```python
from build123d import *

# Parameters (mm, degrees)
SKETCH_1_R      = 4
EXTRUDE_1_DEPTH = 140
EXTRUDE_START   = -20
SKETCH_2_R      = 7.5
EXTRUDE_2_DEPTH = 5
EXTRUDE_START_2 = -15
SKETCH_3_R      = 7.5
EXTRUDE_3_DEPTH = 5


with BuildPart() as part:
    # 草图1 → 凸台-拉伸1 (new, symmetric)
    with BuildSketch(Plane.XY):
        Circle(SKETCH_1_R)
    extrude(amount=EXTRUDE_1_DEPTH, both=True)

    # 草图2 → 凸台-拉伸2 (add)
    with BuildSketch(Plane.XY.offset(140).offset(EXTRUDE_START)):
        Circle(SKETCH_2_R)
    extrude(amount=-EXTRUDE_2_DEPTH)

    # 草图3 → 凸台-拉伸3 (add)
    with BuildSketch(Plane(origin=(0, 0, -140), x_dir=(-1, 0, 0), z_dir=(0, 0, -1)).offset(EXTRUDE_START_2)):
        with Locations(Location((0, 0, 0), (0, 0, 180))):
            Circle(SKETCH_3_R)
    extrude(amount=EXTRUDE_3_DEPTH)


solid = part.part
```
Geometry: final body of the model. Coordinates: model frame, mm. A direction names the side the tool comes from. Coordinates: 2 decimals unless noted, no trailing zeros. Order: outer loops, then holes, each group sorted by start corner. A loop starts at its lowest first (then second) coordinate and runs counter-clockwise, first axis right, second up. Notation, with made-up numbers: M -14,39 L 22,39 A22 ccw 22,68 Z; hole C 44,65 d6. An arc over 180 degrees is marked long. Answer in a Markdown table with one row per item. Add a question column.
Q1. Mould query, pull axis Z, two halves, no side actions, for faces 5 (the flat face through (3, 3, -130)), 6 (the cylindrical face through (4.032, -6.324, -127.465)), 7 (the flat face through (3, -3, 115)). Classes: released by +Z, released by -Z, zero draft, split by the parting line, or undercut.
Q2. Reachability of faces 1 (the cylindrical face through (-0.867, -3.905, 130.14)), 2 (the cylindrical face through (-0.867, -3.905, -134.93)), 3 (the cylindrical face through (-0.867, -3.905, -3.32)), 4 (the flat face through (0, 0, 140)) from +Z, -Z, +X, -X, +Y, -Y: full face, straight path, thin tool, end or side. Return the list, or none.
Q3. Section query A-A on x = 0. Return the cut outline in (y, z), and give its area (3 significant figures).
Q4. Line query: L1, parallel to Z at x = 5.25, y = 0; L2, parallel to Y at x = -0.25, z = -32; L3, parallel to Y at x = -2, z = 59.5. Output: solid intervals per line, ascending.
Q5. Section query C-C on z = -100.5. Return the cut outline in (x, y), and give its area (3 significant figures).
Q6. Contact query for flat-ended pins moving along their axis: P1, Ø6, axis at x = -3, z = 96, coming from the -Y side; P2, Ø1.5, axis at y = -2, z = -12, coming from the -X side. Output: stop coordinate, or through.
Completed:
| question | item | result |
|---|---|---|
| 1 | face 5 | released by -Z |
| 1 | face 6 | zero draft |
| 1 | face 7 | undercut |
| 2 | face 1 | +Z |
| 2 | face 2 | -Z |
| 2 | face 3 | none |
| 2 | face 4 | +Z, +X, -X, +Y, -Y |
| 3 | outline | M -7.5,-130 L -4,-130 L -4,-140 L 4,-140 L 4,-130 L 7.5,-130 L 7.5,-125 L 4,-125 L 4,115 L 7.5,115 L 7.5,120 L 4,120 L 4,140 L -4,140 L -4,120 L -7.5,120 L -7.5,115 L -4,115 L -4,-125 L -7.5,-125 Z |
| 3 | area | 2,310 mm2 |
| 4 | L1 | z = -130 to -125, 115 to 120 |
| 4 | L2 | y = -3.99 to 3.99 |
| 4 | L3 | y = -3.46 to 3.46 |
| 5 | outline | C 0,0 d8 |
| 5 | area | 50.3 mm2 |
| 6 | P1 | stops at y = -4 |
| 6 | P2 | stops at x = -3.8 |
